from build123d import *

# Parameters (mm, degrees)
BASE_TRAPEZOID_SKETCH_W     = 90
BASE_TRAPEZOID_SKETCH_H     = 20
TRAPEZOID_BASE_DEPTH        = 60
CYLINDER_SUPPORT_DEPTH      = 42
SUPPORT_NOTCH_CUT_DEPTH     = 18
SUPPORT_RELIEF_CUT_DEPTH    = 24
THROUGH_PROFILE_CUT_DEPTH   = 60
CYLINDER_SKETCH_40_R        = 20
CYLINDER_40_DEPTH           = 34
CYLINDER_START              = 10
CYLINDER_EXTENSION_SKETCH_R = 20
CYLINDER_EXTENSION_40_DEPTH = 10
FRONT_BORE_SKETCH_16_R      = 8
FRONT_BORE_16_DEPTH         = 10
REAR_START                  = -10
REAR_BORE_SKETCH_R          = 8
REAR_BORE_DEPTH             = 10
SIDE_BLOCKS_DEPTH           = 86
BLOCK_TRIM_SKETCH_W         = 18
BLOCK_TRIM_SKETCH_H         = 35
BLOCK_TRIM_CUT_DEPTH        = 3.7
SLOT_A_SKETCH_W             = 24
SLOT_A_SKETCH_H             = 20
SLOT_A_CUT_DEPTH            = 10
SLOT_B_SKETCH_W             = 24
SLOT_B_SKETCH_H             = 20
SLOT_B_CUT_DEPTH            = 10
FRONT_START                 = 10
FRONT_BORE_FILL_SKETCH_R    = 8
FRONT_BORE_FILL_DEPTH       = 10
REAR_BORE_FILL_SKETCH_R     = 8
REAR_BORE_FILL_DEPTH        = 10
SLOT_B_FLOOR_SKETCH_W       = 24
SLOT_B_FLOOR_SKETCH_H       = 17.320508076
SLOT_B_FLOOR_CUT_DEPTH      = 2
SLOT_A_FLOOR_SKETCH_W       = 24
SLOT_A_FLOOR_SKETCH_H       = 17.320508076
SLOT_A_FLOOR_CUT_DEPTH      = 2
FRONT_BORE_RECUT_SKETCH_R   = 8
FRONT_BORE_RECUT_DEPTH      = 9
REAR_START_2                = -9
REAR_BORE_RECUT_SKETCH_R    = 8
REAR_BORE_RECUT_DEPTH       = 9


with BuildPart() as part:
    # Base Trapezoid Sketch → Trapezoid Base (new body)
    with BuildSketch(Plane.XY):
        with Locations((45, 10)):
            Rectangle(BASE_TRAPEZOID_SKETCH_W, BASE_TRAPEZOID_SKETCH_H)
    extrude(amount=TRAPEZOID_BASE_DEPTH)

    # Support Profile Sketch → Cylinder Support (add)
    with BuildSketch(Plane.XY.offset(60)):
        Polygon((45, 20), (7.272727273, 20), (20, 55), (45, 55), (70, 55), (82.727272727, 20), align=None)
    extrude(amount=-CYLINDER_SUPPORT_DEPTH)

    # Support Notch Sketch → Support Notch Cut (cut)
    with BuildSketch(Plane.XY.offset(60)):
        Polygon((7.272727273, 20), (20, 55), (70, 55), (82.727272727, 20), align=None)
    extrude(amount=-SUPPORT_NOTCH_CUT_DEPTH, mode=Mode.SUBTRACT)

    # Support Relief Sketch → Support Relief Cut (cut)
    with BuildSketch(Plane.XY.offset(42)):
        Polygon((45, 50), (71.818181818, 50), (70, 55), (20, 55), (18.181818182, 50), align=None)
    extrude(amount=-SUPPORT_RELIEF_CUT_DEPTH, mode=Mode.SUBTRACT)

    # Through Profile Sketch → Through Profile Cut (cut)
    with BuildSketch(Plane.XY.offset(60)):
        Polygon((7.272727273, 20), (0, 20), (0, 0), align=None)
        Polygon((90, 20), (82.727272727, 20), (90, 0), align=None)
    extrude(amount=-THROUGH_PROFILE_CUT_DEPTH, mode=Mode.SUBTRACT)

    # Cylinder Sketch Ø40 → Cylinder Ø40 (add)
    with BuildSketch(Plane.XY.offset(42)):
        with Locations((45, 50)):
            Circle(CYLINDER_SKETCH_40_R)
    extrude(amount=-CYLINDER_40_DEPTH)

    # Cylinder Extension Sketch → Cylinder Extension Ø40 (add)
    with BuildSketch(Plane.XY.offset(42).offset(CYLINDER_START)):
        with Locations((45, 50)):
            Circle(CYLINDER_EXTENSION_SKETCH_R)
    extrude(amount=-CYLINDER_EXTENSION_40_DEPTH)

    # Front Bore Sketch Ø16 → Front Bore Ø16 (cut)
    with BuildSketch(Plane.XY.offset(52)):
        with Locations((45, 50)):
            Circle(FRONT_BORE_SKETCH_16_R)
    extrude(amount=-FRONT_BORE_16_DEPTH, mode=Mode.SUBTRACT)

    # Rear Bore Sketch → Rear Bore (cut)
    with BuildSketch(Plane(origin=(0, 0, 8), x_dir=(-1, 0, 0), z_dir=(0, 0, -1)).offset(REAR_START)):
        with Locations(Location((-45, 50, 0), (0, 0, 180))):
            Circle(REAR_BORE_SKETCH_R)
    extrude(amount=REAR_BORE_DEPTH, mode=Mode.SUBTRACT)

    # Side Block Sketch → Side Blocks (add)
    with BuildSketch(Plane(origin=(0, 0, 0), x_dir=(0, 0, -1), z_dir=(1, 0, 0))):
        Polygon((-30, 45), (-39, 45), (-39, 10), (-21, 10), (-21, 45), align=None)
    extrude(amount=SIDE_BLOCKS_DEPTH)

    # Block Trim Sketch → Block Trim Cut (cut)
    with BuildSketch(Plane.ZY):
        with Locations((30, 27.5)):
            Rectangle(BLOCK_TRIM_SKETCH_W, BLOCK_TRIM_SKETCH_H)
    extrude(amount=-BLOCK_TRIM_CUT_DEPTH, mode=Mode.SUBTRACT)

    # Slot A Sketch → Slot A Cut (cut)
    with BuildSketch(Plane(origin=(65, 0, 0), x_dir=(0, 0, -1), z_dir=(1, 0, 0))):
        with Locations((-30, 60)):
            Rectangle(SLOT_A_SKETCH_W, SLOT_A_SKETCH_H)
    extrude(amount=-SLOT_A_CUT_DEPTH, mode=Mode.SUBTRACT)

    # Slot B Sketch → Slot B Cut (cut)
    with BuildSketch(Plane(origin=(25, 0, 0), x_dir=(0, 0, -1), z_dir=(1, 0, 0))):
        with Locations((-30, 60)):
            Rectangle(SLOT_B_SKETCH_W, SLOT_B_SKETCH_H)
    extrude(amount=SLOT_B_CUT_DEPTH, mode=Mode.SUBTRACT)

    # Front Bore Fill Sketch → Front Bore Fill (add)
    with BuildSketch(Plane.XY.offset(42).offset(FRONT_START)):
        with Locations(Location((45, 50, 0), (0, 0, 180))):
            Circle(FRONT_BORE_FILL_SKETCH_R)
    extrude(amount=-FRONT_BORE_FILL_DEPTH)

    # Rear Bore Fill Sketch → Rear Bore Fill (add)
    with BuildSketch(Plane(origin=(0, 0, 18), x_dir=(-1, 0, 0), z_dir=(0, 0, -1))):
        with Locations((-45, 50)):
            Circle(REAR_BORE_FILL_SKETCH_R)
    extrude(amount=REAR_BORE_FILL_DEPTH)

    # Slot B Floor Sketch → Slot B Floor Cut (cut)
    with BuildSketch(Plane.ZY.offset(-35)):
        with Locations((30, 58.660254038)):
            Rectangle(SLOT_B_FLOOR_SKETCH_W, SLOT_B_FLOOR_SKETCH_H)
    extrude(amount=-SLOT_B_FLOOR_CUT_DEPTH, mode=Mode.SUBTRACT)

    # Slot A Floor Sketch → Slot A Floor Cut (cut)
    with BuildSketch(Plane(origin=(55, 0, 0), x_dir=(0, 0, -1), z_dir=(1, 0, 0))):
        with Locations((-30, 58.660254038)):
            Rectangle(SLOT_A_FLOOR_SKETCH_W, SLOT_A_FLOOR_SKETCH_H)
    extrude(amount=-SLOT_A_FLOOR_CUT_DEPTH, mode=Mode.SUBTRACT)

    # Front Bore Recut Sketch → Front Bore Recut (cut)
    with BuildSketch(Plane.XY.offset(52)):
        with Locations((45, 50)):
            Circle(FRONT_BORE_RECUT_SKETCH_R)
    extrude(amount=-FRONT_BORE_RECUT_DEPTH, mode=Mode.SUBTRACT)

    # Rear Bore Recut Sketch → Rear Bore Recut (cut)
    with BuildSketch(Plane(origin=(0, 0, 8), x_dir=(-1, 0, 0), z_dir=(0, 0, -1)).offset(REAR_START_2)):
        with Locations(Location((-45, 50, 0), (0, 0, 180))):
            Circle(REAR_BORE_RECUT_SKETCH_R)
    extrude(amount=REAR_BORE_RECUT_DEPTH, mode=Mode.SUBTRACT)


solid = part.part
CAD build for the part. Positions are in the model's coordinates, mm. A direction names the side the tool comes from. Coordinates: 2 decimals unless noted, no trailing zeros. Write each loop counter-clockwise with the first axis right and the second up, starting at its lowest first coordinate (ties: lowest second). Pieces come first, ordered by that corner, then holes. Notation, with made-up numbers: M -20,47 L 32,47 A19 ccw 32,70 Z; hole C 43,24 d1. An arc over 180 degrees is marked long. Answer as a JSON object with one key per item and string values. Group by question number.
1) Pin check, flat tips, straight feed: pin 1 Ø14.5 at (x, z) = (48.5, 9.5) entering from +Y; pin 2 Ø4 at (x, y) = (7.5, 25) entering from -Z; pin 3 Ø12 at (x, y) = (36, 50.5) entering from +Z. Stop position of each tip, or through.
2) Saw through at D-D (z = 24). Write the cut outline in (x, y).
3) Mould opens along Y. For faces 6 (the face through (9, 32, 39)), 7 (the face through (10, 45, 30)), 8 (the face through (44, 29, 42)), 9 (the face through (53, 59, 30)) say: +Y half, -Y half, draft (parallel to the pull), parting line (faces both ways), or undercut.
4) Saw through at B-B (x = 61). Write the cut outline in (y, z).
5) Wall check: line 1 (Y direction, x = 45, z = 48); line 2 (Y direction, x = 31.5, z = 34.5); line 3 (Z direction, x = 52, y = 37). Give the ranges that are in metal, low to high. Write a range as from..to.
6) Saw through at A-A (z = 44.5). Write the cut outline in (x, y).
7) Saw through at C-C (y = 35.5). Write the cut outline in (x, z).
8) Tool access for faces 1 (the face through (39.1, 55.4, 47.6)), 2 (the face through (32, 57, 18)), 3 (the face through (7, 35, 21)), 4 (the face through (45, 41, 8)), 5 (the face through (3.7, 28, 30)): list every direction of +Z, -Z, +X, -X, +Y, -Y with a clear straight run to the whole face (end or side of a thin tool).
Values follow:
{
 "1": {"pin 1": "stops at y = 70", "pin 2": "stops at z = 18", "pin 3": "stops at z = 52"},
 "2": {"outline": "M 0,0 L 90,0 L 86,11 L 86,45 L 73.64,45 L 71.82,50 L 53,50 L 53,67.32 L 55,67.32 A20 ccw 35,67.32 L 37,67.32 L 37,50 L 18.18,50 L 16.36,45 L 3.7,45 L 3.7,10 L 3.64,10 Z"},
 "3": {"face 6": "draft", "face 7": "+Y half", "face 8": "undercut", "face 9": "undercut"},
 "4": {"outline": "M 0,0 L 20,0 L 20,18 L 38,18 L 38,8 L 62,8 L 62,18 L 50,18 L 50,42 L 62,42 L 62,52 L 38,52 L 38,42 L 20,42 L 20,60 L 0,60 Z"},
 "5": {"line 1": "y = 0..20, 30..42, 58..70", "line 2": "y = 0..50", "line 3": "z = 8..52"},
 "6": {"outline": "M 0,0 L 90,0 L 82.73,20 L 7.27,20 Z; C 45,50 d40; hole C 45,50 d16"},
 "7": {"outline": "M 3.7,21 L 12.91,21 L 12.91,18 L 31.23,18 L 31.23,8 L 58.77,8 L 58.77,18 L 77.09,18 L 77.09,21 L 86,21 L 86,39 L 77.09,39 L 77.09,42 L 58.77,42 L 58.77,52 L 31.23,52 L 31.23,42 L 12.91,42 L 12.91,39 L 3.7,39 Z"},
 "8": {"face 1": "+Z", "face 2": "-X", "face 3": "-Z, -X, +Y", "face 4": "-Z, +X, -X, +Y", "face 5": "+Z, -Z, -X, +Y"}
}
